from build123d import *

# Parameters (mm, degrees)
SKETCH1_R = 2


with BuildPart() as part:
    # Sweep1: sweep along a curve in space
    with BuildLine() as sweep1_path:
        Line((-50.19826571, 33.779851644, 68.304462045), (-50.190924205, 36.164146317, 69.680554329))
        ThreePointArc((-50.190924205, 36.164146317, 69.680554329), (-50.168295566, 45.270129978, 70.877966766), (-50.158922477, 52.555749547, 65.285748364))
        Line((-50.158922477, 52.555749547, 65.285748364), (-50.158922477, 66.080807741, 41.85147393))
        ThreePointArc((-50.158922477, 73.043553961, 15.8582869), (-50.158922477, 71.272714796, 29.313077932), (-50.158922477, 66.080807741, 41.85147393))
        Line((-50.158922477, 73.043553961, 15.8582869), (-50.158922477, 73.043553961, 12.109558404))
        ThreePointArc((-62.158922477, 73.043553961, 0.109558404), (-53.673641103, 73.043553961, 3.62427703), (-50.158922477, 73.043553961, 12.109558404))
        Line((-103.577768148, 73.043553961, 0.109558404), (-62.158922477, 73.043553961, 0.109558404))
        ThreePointArc((-103.577768148, 73.043553961, 0.109558404), (-107.820408835, 71.286194648, 0.109558404), (-109.577768148, 67.043553961, 0.109558404))
        Line((-109.577768148, 64.263552475, 0.109558404), (-109.577768148, 67.043553961, 0.109558404))
        ThreePointArc((-109.577768148, 64.263552475, 0.109558404), (-111.335127461, 60.020911788, 0.109558404), (-115.577768148, 58.263552475, 0.109558404))
        Line((-122.59826571, 58.263552475, 0.109558404), (-115.577768148, 58.263552475, 0.109558404))
    # Sketch1 → Sweep1 (sweep)
    with BuildSketch(Plane(origin=(-122.59826571, 0, 0), x_dir=(0, 0, -1), z_dir=(1, 0, 0))):
        with Locations((-0.109558404, 58.263552475)):
            Circle(SKETCH1_R)
    sweep(path=sweep1_path.line)


solid = part.part
For this review, take the finished solid that the model builds, in its own axes (mm). A direction names the side the tool comes from. Round coordinates to 2 decimals unless told otherwise and drop trailing zeros. Write each loop counter-clockwise with the first axis right and the second up, starting at its lowest first coordinate (ties: lowest second). Pieces come first, ordered by that corner, then holes. Notation, with made-up numbers: M 42,69 L 51,69 A3 cw 51,73 Z; hole C 80.25,50.25 d5. An arc over 180 degrees is marked long. Write item = value, one per line. Start each with the question number.
(1) Clearance check with a flat-ended pin moving along its axis: pin 1 Ø2 at (y, z) = (61, 46) entering from -X. State where the tip first meets the part, or that it passes through.
(2) For faces 1 (the face through (-83.158, 74.996, 0.543)), 2 (the face through (-119.14, 60.04, -0.81)), list the 3-axis set-ups (+Z, -Z, +X, -X, +Y, -Y) from which the entire face can be reached by the end or side of a thin tool; tool diameter is ignored.
(3) We need section A-A (x = -102.5). Give the boundary of the cut face in (y, z).
(4) For line 1 along X through (y, z) = (55, 61); line 2 along X through (y, z) = (73.5, 9), list the stretches that pass through material, from the lowest coordinate up.
(5) The part is to be moulded in two halves that separate along Z. For faces 3 (the face through (-122.598, 58, 0)), 4 (the face through (-50.592, 74.996, 13.958)), 5 (the face through (-111.53, 65.63, 0.54)), say which applies: +Z half, -Z half, draft (parallel to the pull), parting line (faces both ways), or undercut.
Results found:
q1.pin_1 = -51.66
q2.face_1 = none
q2.face_2 = -X
q3.outline = C 73.04,0.11 d4
q4.line_1 = -52.16 to -48.16
q4.line_2 = -52.6 to -48.56
q5.face_3 = draft
q5.face_4 = undercut
q5.face_5 = parting line
